The figure shows three views and two pictorial views of one solid part (mm, origin at its lowest corner). Answer the questions. A direction names the side the tool comes from. Coordinates: 2 decimals unless noted, no trailing zeros. Order: outer loops, then holes, each group sorted by start corner. A loop starts at its lowest first (then second) coordinate and runs counter-clockwise, first axis right, second up. Notation, with made-up numbers: (-14, 28.5) -> (-1, 28.5) arc R10 cw to (-1, 41.5) -> close; hole circle Ø5 at (57.5, -35). An arc over 180 degrees is marked (long way). Return JSON: item names as keys, results as strings. Group by question number.
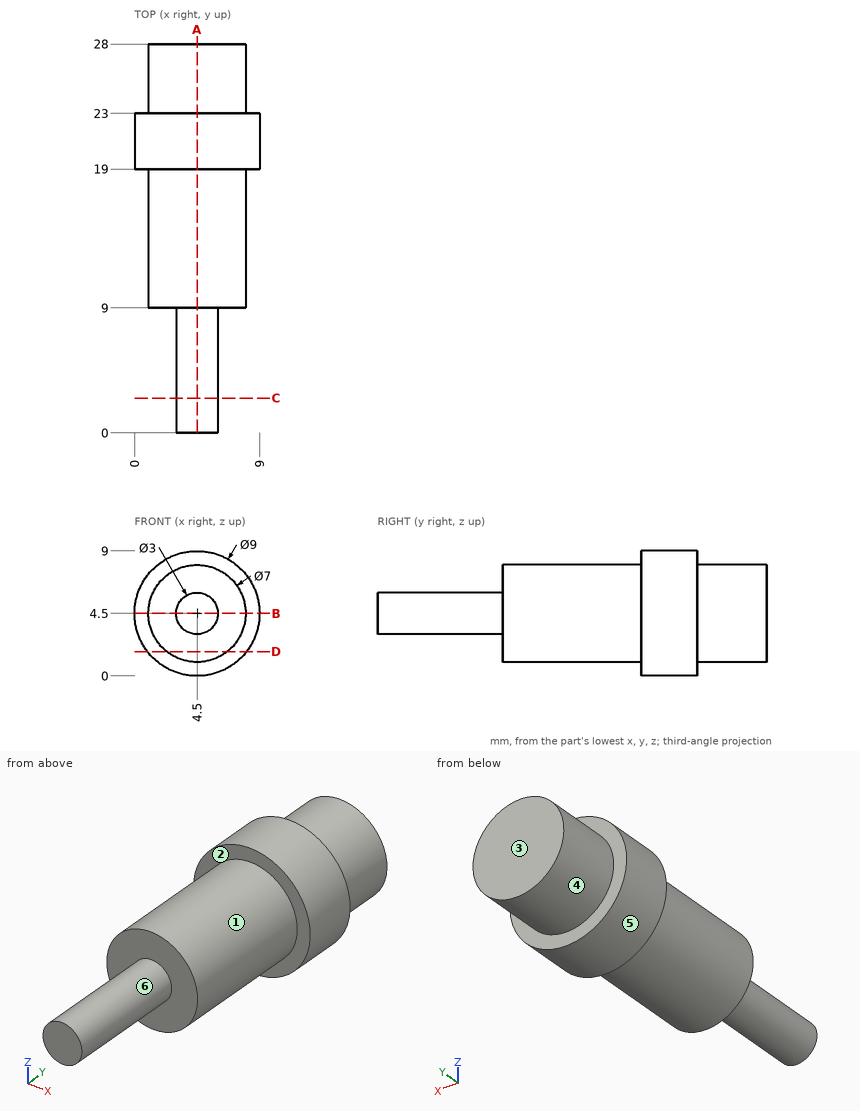
1. Straight lines are drawn through the part: L1, parallel to Y at x = 0.5, z = 3.75; L2, parallel to Y at x = 3, z = 4; L3, parallel to Z at x = 6.5, y = 10. For each, find the intervals that lie inside material, in ascending order.
2. Find section B-B on z = 4.5. Determine the outline of the cut face in (x, y).
3. Find section C-C on y = 2.5. Determine the outline of the cut face in (x, z).
4. Find section A-A on x = 4.5. Determine the outline of the cut face in (y, z).
5. Which of the six approach directions +Z, -Z, +X, -X, +Y, -Y give full straight-line access (tool end or side, diameter ignored) to the marked faces 4, 5 and 6?
6. For a pull along Y with two mould halves and no side action, classify the marked faces 1, 2 and 3 as released by +Y, released by -Y, zero draft, split by the parting line, or undercut.
7. Given pin 1 (4 mm diameter, centred on x = 7.5, z = 6.5, fed in from -Y); pin 2 (2.5 mm diameter, centred on x = 4.5, z = 6.5, fed in from -Y); pin 3 (2 mm diameter, centred on x = 4.5, y = 16, fed in from -Z); pin 4 (5 mm diameter, centred on y = 10.5, z = 7, fed in from +X), each flat-ended and moving along its own axis, determine where each tip first touches the part or whether it passes through.
8. Find section D-D on z = 1.75. Determine the outline of the cut face in (x, y).
Result:
{
 "1": {"L1": "19 to 23", "L2": "9 to 28", "L3": "1.63 to 7.37"},
 "2": {"outline": "(0, 19) -> (1, 19) -> (1, 9) -> (3, 9) -> (3, 0) -> (6, 0) -> (6, 9) -> (8, 9) -> (8, 19) -> (9, 19) -> (9, 23) -> (8, 23) -> (8, 28) -> (1, 28) -> (1, 23) -> (0, 23) -> close"},
 "3": {"outline": "circle Ø3 at (4.5, 4.5)"},
 "4": {"outline": "(0, 3) -> (9, 3) -> (9, 1) -> (19, 1) -> (19, 0) -> (23, 0) -> (23, 1) -> (28, 1) -> (28, 8) -> (23, 8) -> (23, 9) -> (19, 9) -> (19, 8) -> (9, 8) -> (9, 6) -> (0, 6) -> close"},
 "5": {"face 4": "+Y", "face 5": "+Y, -Y", "face 6": "-Y"},
 "6": {"face 1": "zero draft", "face 2": "released by -Y", "face 3": "released by +Y"},
 "7": {"pin 1": "y = 9", "pin 2": "y = 0", "pin 3": "z = 1", "pin 4": "x = 8"},
 "8": {"outline": "(0.94, 19) -> (2.33, 19) -> (2.33, 9) -> (6.67, 9) -> (6.67, 19) -> (8.06, 19) -> (8.06, 23) -> (6.67, 23) -> (6.67, 28) -> (2.33, 28) -> (2.33, 23) -> (0.94, 23) -> close"}
}
